Geometry: final body of the model. Coordinates: model frame, mm. Face numbers are marked on the shaded views. Coordinates: 2 decimals unless noted, no trailing zeros. Write each loop counter-clockwise with the first axis right and the second up, starting at its lowest first coordinate (ties: lowest second). Pieces come first, ordered by that corner, then holes. Notation, with made-up numbers: (1.5, -32.5) - (38.5, -32.5) arc R10 cw to (38.5, -16.5) - close; hole circle Ø4 at (3.25, 22). An arc over 180 degrees is marked (long way). Answer as a JSON object with one key per item and string values. Group by question number.
Item 1: Mould query, pull axis X, two halves, no side actions, for the marked faces 1, 2 and 3. Classes: pulls with the +X half, pulls with the -X half, needs draft (parallel to the pull), parting line crosses it, or undercut.
Item 2: Section C-C on x = -578.5. Return loops of the section in (y, z), and give its area (3 significant figures).
Item 3: Line query: line 1 along Y through (x, z) = (-623, 9.5); line 2 along X through (y, z) = (-84, 15.5); line 3 along Y through (x, z) = (-612, 6.5). Output: solid intervals per line, ascending. Write a range as from..to.
Item 4: Section D-D on y = -110. Return loops of the section in (x, z).
Item 5: Section A-A on y = -90. Return loops of the section in (x, z).
Item 6: Section B-B on z = 9.25. State how many separate pieces and enclosed holes the cut face has, and give its area (3 significant figures).
Item 7: First-contact query: pin 1 Ø12 at (y, z) = (-79, 21.5) entering from -X; pin 2 Ø5.5 at (x, z) = (-642.5, 16.5) entering from +Y; pin 3 Ø1.5 at (y, z) = (-131.5, 10.5) entering from -X; pin 4 Ø10 at (y, z) = (-88, 5) entering from -X. Flat tips, straight axial feed; report the tip coordinate or a pass-through.
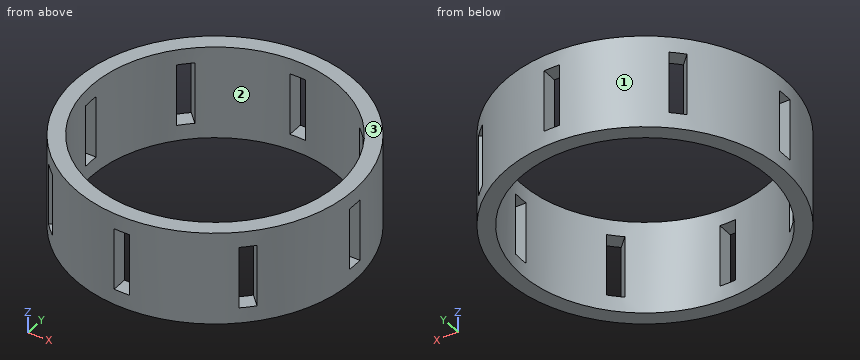
```python
from build123d import *

# Parameters (mm, degrees)
SKETCH1_R           = 45
SKETCH1_R_2         = 40
BOSS_EXTRUDE1_DEPTH = 30
SKETCH2_W           = 5
SKETCH2_H           = 20
CUT_EXTRUDE1_DEPTH  = 660.545773414
CIRPATTERN1_COUNT   = 8


with BuildPart() as part:
    # Sketch1 → Boss-Extrude1 (new body)
    with BuildSketch(Plane.XY):
        with Locations((-599.884196758, -90)):
            Circle(SKETCH1_R)
        with Locations((-599.884196758, -90)):
            Circle(SKETCH1_R_2, mode=Mode.SUBTRACT)
    extrude(amount=BOSS_EXTRUDE1_DEPTH)

    # Sketch2 → Cut-Extrude1 (cut, symmetric)
    with BuildSketch(Plane(origin=(0, 0, 0), x_dir=(1, 0, 0), z_dir=(0, 1, 0))):
        with Locations((-599.884196758, -15)):
            Rectangle(SKETCH2_W, SKETCH2_H)
    cut_extrude1 = extrude(amount=CUT_EXTRUDE1_DEPTH, both=True, mode=Mode.SUBTRACT)

    # CirPattern1: Cut-Extrude1 ×8 about axis
    cirpattern1_axis = Axis((-599.884196758, -90, 0), (0, 0, 1))
    for i in range(1, CIRPATTERN1_COUNT):
        add(cut_extrude1.rotate(cirpattern1_axis, i * 360 / CIRPATTERN1_COUNT), mode=Mode.SUBTRACT)


solid = part.part
```
Checks:
{
 "1": {"face 1": "parting line crosses it", "face 2": "undercut", "face 3": "needs draft"},
 "2": {"outline": "(-129.59, 0) - (-123.8, 0) - (-123.8, 30) - (-129.59, 30) - close; (-56.2, 0) - (-50.41, 0) - (-50.41, 30) - (-56.2, 30) - close", "area": "347 mm^2"},
 "3": {"line 1": "-128.61..-122.64, -57.36..-51.39", "line 2": "-644.48..-639.43, -560.34..-555.29", "line 3": "-133.34..-128.12, -51.88..-46.66"},
 "4": {"outline": "(-640.2, 0) - (-634.53, 0) - (-634.53, 30) - (-640.2, 30) - close; (-565.24, 0) - (-559.57, 0) - (-559.57, 30) - (-565.24, 30) - close"},
 "5": {"outline": "(-644.88, 0) - (-639.88, 0) - (-639.88, 5) - (-644.88, 5) - close; (-644.88, 25) - (-639.88, 25) - (-639.88, 30) - (-644.88, 30) - close; (-559.88, 0) - (-554.88, 0) - (-554.88, 5) - (-559.88, 5) - close; (-559.88, 25) - (-554.88, 25) - (-554.88, 30) - (-559.88, 30) - close"},
 "6": {"separate pieces": "8", "enclosed holes": "0", "area": "1,140 mm^2"},
 "7": {"pin 1": "x = -644.61", "pin 2": "y = -69.13", "pin 3": "x = -618.97", "pin 4": "x = -644.88"}
}
